Part model, mm, in its own coordinate system. Give positions to 0.01 mm unless a question says otherwise; leave off trailing zeros. Loops run counter-clockwise (first coordinate to the right, second up) from the corner with the lowest first, then second, coordinate; pieces in that order, holes last. Notation, with made-up numbers: (78, -24.5) -> (137, -24.5) arc R17 cw to (137, -19.5) -> close; hole circle Ø11 at (24.25, -22.75). An arc over 180 degrees is marked (long way). One line per question, with ' | ' between items.
```python
from build123d import *

# Parameters (mm, degrees)
SKETCH1_W           = 30
SKETCH1_H           = 30
BOSS_EXTRUDE1_DEPTH = 4
SKETCH3_R           = 7
CUT_EXTRUDE2_DEPTH  = 43.614551505


with BuildPart() as part:
    # Sketch1 → Boss-Extrude1 (new body)
    with BuildSketch(Plane(origin=(0, 0, 0), x_dir=(1, 0, 0), z_dir=(0, 1, 0))):
        with Locations((15, -15)):
            Rectangle(SKETCH1_W, SKETCH1_H)
    extrude(amount=BOSS_EXTRUDE1_DEPTH)

    # Sketch3 → Cut-Extrude2 (cut, through all)
    with BuildSketch(Plane(origin=(0, 4, 0), x_dir=(1, 0, 0), z_dir=(0, 1, 0))):
        with Locations(Location((15, -15, 0), (0, 0, 270))):
            Circle(SKETCH3_R)
    extrude(amount=-CUT_EXTRUDE2_DEPTH, mode=Mode.SUBTRACT)


solid = part.part
```
1) Saw through at B-B (x = 15). Give the cut face in (y, z), and give its area (3 significant figures).
Found:
outline: (0, 0) -> (4, 0) -> (4, 8) -> (0, 8) -> close; (0, 22) -> (4, 22) -> (4, 30) -> (0, 30) -> close | area: 64.0 mm2
2) Saw through at A-A (z = 15). Give the cut face in (x, y), and give its area (3 significant figures).
Found:
outline: (0, 0) -> (8, 0) -> (8, 4) -> (0, 4) -> close; (22, 0) -> (30, 0) -> (30, 4) -> (22, 4) -> close | area: 64.0 mm2
3) Drill centre lines: line 1 (X direction, y = 1.7, z = 15); line 2 (X direction, y = 3.1, z = 11.75); line 3 (Z direction, x = 8.75, y = 3). Where is each one in solid material? Low to high.
Found:
line 1: 0 to 8, 22 to 30 | line 2: 0 to 8.8, 21.2 to 30 | line 3: 0 to 11.85, 18.15 to 30
4) Pull direction Z, two halves, no side cores. Call faces 1 (the flat face through (8, 0, 18)), 2 (the flat face through (15, 2, 0)), 3 (the cylindrical face through (10.741, 2.028, 9.445)), 4 (the flat face through (15, 2, 30)): pulls with the +Z half, pulls with the -Z half, needs draft (parallel to the pull), parting line crosses it, or undercut.
Found:
face 1: needs draft | face 2: pulls with the -Z half | face 3: undercut | face 4: pulls with the +Z half
5) Saw through at C-C (y = 1.15). Give the cut face in (x, z).
Found:
outline: (0, 0) -> (30, 0) -> (30, 30) -> (0, 30) -> close; hole circle Ø14 at (15, 15)
